Input: part model. Units: mm. Frame: model coordinates. Face numbers are marked on the shaded views. A direction names the side the tool comes from. Round coordinates to 2 decimals unless told otherwise and drop trailing zeros. Loops run counter-clockwise (first coordinate to the right, second up) from the corner with the lowest first, then second, coordinate; pieces in that order, holes last.
(1) Line query: line 1 (X direction, y = 0, z = -5.35); line 2 (Y direction, x = 4.5, z = -6.75). Output: solid intervals per line, ascending.
(2) First-contact query: pin 1 Ø1 at (y, z) = (1.5, -6) entering from -X. Flat tip, straight axial feed; report the tip coordinate or a pass-through.
(3) Cut plane C-C, the plane z = -5.05. Output: boundary loops of the cut face in (x, y), and give its area (3 significant figures).
(4) Cut plane A-A, the plane x = -2. Output: boundary loops of the cut face in (y, z).
(5) Cut plane B-B, the plane y = 3.25. Output: boundary loops of the cut face in (x, z).
(6) Cut plane D-D, the plane x = 6.5. Output: boundary loops of the cut face in (y, z), and give its area (3 significant figures).
(7) Access query for the marked faces 1 and 2. Directions: +Z, -Z, +X, -X, +Y, -Y. A direction counts if a zero-diameter tool reaches every point of the face in a straight line with its end or side. Return the directions, or none.
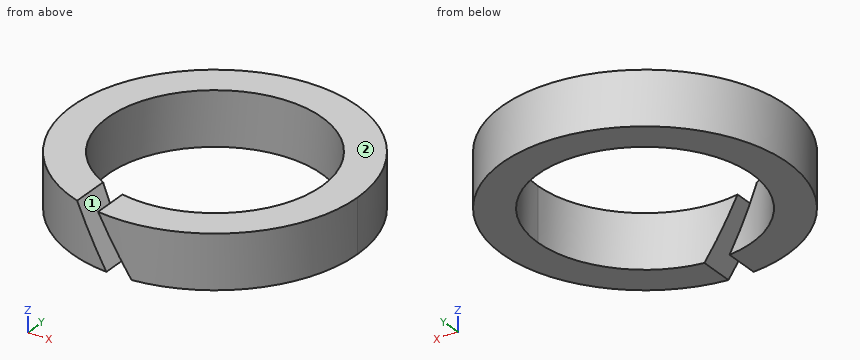
from build123d import *

# Parameters (mm, degrees)
SKETCH1_W          = 2
SKETCH1_H          = 3
CUT_EXTRUDE1_DEPTH = 23


with BuildPart() as part:
    # Sketch1 → Revolve1 (revolve)
    with BuildSketch(Plane(origin=(0, 0, 0), x_dir=(1, 0, 0), z_dir=(0, 1, 0))):
        with Locations((7, 5.564714504)):
            Rectangle(SKETCH1_W, SKETCH1_H)
    revolve(axis=Axis((0, 0, 0), (0, 0, -1)))

    # Sketch2 → Cut-Extrude1 (cut)
    with BuildSketch(Plane(origin=(0, 0, 0), x_dir=(1, 0, 0), z_dir=(0, 1, 0))):
        Polygon((-3.27585187, 3.09237347), (2.379628245, 11.930992665), (3.38205654, 11.289578756), (-2.273423575, 2.450959561), align=None)
    extrude(amount=-CUT_EXTRUDE1_DEPTH, mode=Mode.SUBTRACT)


solid = part.part
Reported:
1. line 1: x = -8 to -6, 6 to 8
1. line 2: y = -6.61 to -3.97, 3.97 to 6.61
2. pin 1: stops at x = -7.94
3. outline: (-2.02, -7.74) - (-2.02, -5.65) arc R6 cw (long way) to (-0.61, -5.97) - (-0.61, -7.98) arc R8 ccw (long way) to start
3. area: 85.1 mm2
4. outline: (-7.75, -7.06) - (-5.66, -7.06) - (-5.66, -5.09) - (-7.75, -5.09) - close; (5.66, -7.06) - (7.75, -7.06) - (7.75, -4.06) - (5.66, -4.06) - close
5. outline: (-7.31, -7.06) - (-5.04, -7.06) - (-5.04, -4.06) - (-7.31, -4.06) - close; (5.04, -7.06) - (7.31, -7.06) - (7.31, -4.06) - (5.04, -4.06) - close
6. outline: (-4.66, -7.06) - (4.66, -7.06) - (4.66, -4.06) - (-4.66, -4.06) - close
6. area: 28.0 mm2
7. face 1: -Y
7. face 2: +Z, +X, -X, +Y, -Y
